```python
from build123d import *

# Parameters (mm, degrees)
SKETCH_1_R        = 1
EXTRUDE_967_DEPTH = 1


with BuildPart() as part:
    # 草图1 → Extrude 967 (new body)
    with BuildSketch(Plane.XY):
        with BuildLine():
            Line((-4.368765084, -10.547131916), (-5.338433881, -12.888119479))
            ThreePointArc((-5.338433881, -12.888119479), (0, 13.95), (5.338433881, -12.888119479))
            Line((5.338433881, -12.888119479), (4.368765084, -10.547131916))
            ThreePointArc((4.368765084, -10.547131916), (5.045920823, -8.160133818), (7.524722821, -8.268947735))
            ThreePointArc((7.524722821, -8.268947735), (8.418733826, -8.556288298), (9.245939718, -8.111821553))
            ThreePointArc((9.245939718, -8.111821553), (0, 11.15), (-9.245939718, -8.111821553))
            ThreePointArc((-9.245939718, -8.111821553), (-8.418733826, -8.556288298), (-7.524722821, -8.268947735))
            ThreePointArc((-7.524722821, -8.268947735), (-5.045920823, -8.160133818), (-4.368765084, -10.547131916))
        make_face()
        with Locations((-6.298089329, -9.978680815)):
            Circle(SKETCH_1_R, mode=Mode.SUBTRACT)
        with Locations(Location((6.298089329, -9.978680815, 0), (0, 0, 180))):
            Circle(SKETCH_1_R, mode=Mode.SUBTRACT)
    extrude(amount=EXTRUDE_967_DEPTH)


solid = part.part
```
Model file for the job. Use its own axes, mm. A direction names the side the tool comes from. Coordinates: 2 decimals unless noted, no trailing zeros. Order: outer loops, then holes, each group sorted by start corner. A loop starts at its lowest first (then second) coordinate and runs counter-clockwise, first axis right, second up. Notation, with made-up numbers: (37, 51) -> (78, 51) arc R15 cw to (78, 68) -> close; hole circle Ø5 at (-21.75, 86). An arc over 180 degrees is marked (long way). Return JSON: item names as keys, results as strings.
Item 1: Wall check: line 1 along Y through (x, z) = (5.75, 0.4); line 2 along X through (y, z) = (6, 0.15); line 3 along Y through (x, z) = (-5.5, 0.6). Give the ranges that are in metal, low to high. Write a range as from..to.
Model answer:
{"line 1": "y = -12.71..-10.82, -9.14..-7.84, 9.66..12.71", "line 2": "x = -12.59..-9.77, 9.77..12.59", "line 3": "y = -12.82..-10.58, -9.38..-7.91, 9.8..12.82"}
Item 2: 3-axis set-ups, long thin cutter, end or side, ignore diameter. For faces 1 (the face through (-8.432, -8.555, 0.493)), 2 (the face through (4, 11, 0)), 3 (the face through (4.86, -11.73, 0.49)): which of +Z, -Z, +X, -X, +Y, -Y reach the whole face in a straight line?
Model answer:
{"face 1": "+Z, -Z", "face 2": "-Z, +X, -X, +Y, -Y", "face 3": "+Z, -Z, -Y"}
Item 3: Slice it at C-C (x = -6.5). Write the cut outline in (y, z), then the cut area to 3 significant figures.
Model answer:
{"outline": "(-12.34, 0) -> (-10.96, 0) -> (-10.96, 1) -> (-12.34, 1) -> close; (-9, 0) -> (-7.8, 0) -> (-7.8, 1) -> (-9, 1) -> close; (9.21, 0) -> (12.34, 0) -> (12.34, 1) -> (9.21, 1) -> close", "area": "5.72 mm²"}
Item 4: Pin check, flat tip, straight feed: P1, Ø14, axis at x = 0, y = -0.7, coming from the -Z side. Stop position of the tip, or through.
Model answer:
{"P1": "passes through"}
Item 5: Mould opens along Y. For faces 4 (the face through (-4.847, -11.701, 0.493)), 5 (the face through (0.373, 11.144, 0.493)), 6 (the face through (4, 11, 1)), 7 (the face through (-0.54, 13.94, 0.49)) say: pulls with the +Y half, pulls with the -Y half, needs draft (parallel to the pull), parting line crosses it, or undercut.
Model answer:
{"face 4": "pulls with the -Y half", "face 5": "undercut", "face 6": "needs draft", "face 7": "parting line crosses it"}
Item 6: Slice it at A-A (x = 8). Write the cut outline in (y, z).
Model answer:
{"outline": "(-11.43, 0) -> (-8.52, 0) -> (-8.52, 1) -> (-11.43, 1) -> close; (8.04, 0) -> (11.43, 0) -> (11.43, 1) -> (8.04, 1) -> close"}
Item 7: Slice it at B-B (y = 0). Write the cut outline in (x, z).
Model answer:
{"outline": "(-13.95, 0) -> (-11.83, 0) -> (-11.83, 1) -> (-13.95, 1) -> close; (11.83, 0) -> (13.95, 0) -> (13.95, 1) -> (11.83, 1) -> close"}
Item 8: Slice it at D-D (z = 0.8). Write the cut outline in (x, y).
Model answer:
{"outline": "(-9.25, -8.11) arc R11.85 cw (long way) to (9.25, -8.11) arc R1.2 cw to (7.52, -8.27) arc R2 ccw to (4.37, -10.55) -> (5.34, -12.89) arc R13.95 ccw (long way) to (-5.34, -12.89) -> (-4.37, -10.55) arc R2 ccw to (-7.52, -8.27) arc R1.2 cw to start; hole circle Ø2 at (-6.3, -9.98); hole circle Ø2 at (6.3, -9.98)"}
